For this review, take the finished solid that the model builds, in its own axes (mm). A direction names the side the tool comes from. Give positions to 0.01 mm unless a question says otherwise; leave off trailing zeros. Order: outer loops, then holes, each group sorted by start corner. A loop starts at its lowest first (then second) coordinate and runs counter-clockwise, first axis right, second up. Notation, with made-up numbers: (43, 53.25) -> (54, 53.25) arc R5 ccw to (54, 60.25) -> close; hole circle Ø10 at (-22.5, -24.5). An arc over 180 degrees is marked (long way). Return JSON: item names as keys, results as strings. Group by question number.
1) Add section D-D (x = 123). Give the boundary of the cut face in (y, z).
2) Add section B-B (x = -110). Give the boundary of the cut face in (y, z), then the cut area to 3 significant figures.
3) Add section A-A (z = 196). Give the boundary of the cut face in (x, y), then the cut area to 3 significant figures.
4) To check wall thickness, follow line 1 along Z through (x, y) = (18.5, 234); line 2 along Z through (x, y) = (100.5, 329); line 3 along Y through (x, z) = (327.5, 166). State the ranges of each line that lie inside material, in increasing order.
5) The part is to be moulded in two halves that separate along X. For faces 4 (the face through (211, 309, 0)), 5 (the face through (104.15, -180.39, 138.19)), 6 (the face through (487.348, 444.111, 118.11)), say which applies: released by +X, released by -X, zero draft, split by the parting line, or undercut.
6) Add section C-C (y = 546.5). Give the boundary of the cut face in (x, z), then the cut area to 3 significant figures.
7) Insertion check: P1, Ø12, axis at x = 323, z = 144.5, coming from the +Y side; P2, Ø16, axis at y = 202.5, z = 289, coming from the -X side; P3, Ø2, axis at x = 314.5, z = 206, coming from the -Y side. Each pin has a flat end and moves straight along its axis. Give the tip position at first contact, or say it passes through.
8) For faces 1 (the face through (-108, 345, 148)), 2 (the face through (-111, 424, 270)), 3 (the face through (0, 474, 148)), list the 3-axis set-ups (+Z, -Z, +X, -X, +Y, -Y) from which the entire face can be reached by the end or side of a thin tool; tool diameter is ignored.
from build123d import *

# Parameters (mm, degrees)
BOSS_EXTRUDE1_DEPTH = 300
CUT_EXTRUDE2_START  = -20
CUT_EXTRUDE2_DEPTH  = 260
SKETCH3_R           = 25
CUT_EXTRUDE3_DEPTH  = 932.86425071
SKETCH4_R           = 15
SKETCH4_W           = 55
SKETCH4_H           = 160
CUT_EXTRUDE4_DEPTH  = 932.86425071
SKETCH5_R           = 15
SKETCH5_W           = 160
SKETCH5_H           = 55
CUT_EXTRUDE5_DEPTH  = 1055.203993494
SKETCH7_R           = 15
SKETCH7_W           = 55
SKETCH7_H           = 160
CUT_EXTRUDE6_DEPTH  = 954.980428731
CUT_EXTRUDE7_REACH  = 933.864
SKETCH8_R           = 110
SKETCH9_W           = 270
SKETCH9_H           = 190
CUT_EXTRUDE8_DEPTH  = 100
CIRPATTERN1_COUNT   = 3


with BuildPart() as part:
    # Sketch1 → Boss-Extrude1 (new body)
    with BuildSketch(Plane.XY):
        Polygon((0, 0), (0, 345), (-220, 345), (-220, 600), (0, 600), (298.778764306, 427.5), (408.778764306, 618.025588833), (629.615242271, 490.525588833), (519.615242271, 300), (220.836477965, 127.5), (330.836477965, -63.025588833), (110, -190.525588833), align=None)
    extrude(amount=BOSS_EXTRUDE1_DEPTH)

    # Sketch2 → Cut-Extrude2 (cut)
    with BuildSketch(Plane(origin=(0, 0, 0), x_dir=(-1, 0, 0), z_dir=(0, 0, -1)).offset(CUT_EXTRUDE2_START)):
        Polygon((0, 600), (0, 0), (-519.615242271, 300), align=None)
    extrude(amount=-CUT_EXTRUDE2_DEPTH, mode=Mode.SUBTRACT)

    # Sketch3 → Cut-Extrude3 (cut, through all)
    with BuildSketch(Plane(origin=(0, 0, 0), x_dir=(-1, 0, 0), z_dir=(0, 0, -1))):
        with Locations((-173.205080757, 300)):
            Circle(SKETCH3_R)
    extrude(amount=-CUT_EXTRUDE3_DEPTH, mode=Mode.SUBTRACT)

    # Sketch4 → Cut-Extrude4 (cut, through all)
    with BuildSketch(Plane(origin=(0, 0, 0), x_dir=(0, 0, 1), z_dir=(-0.866025403784456, -0.4999999999999701, 0))):
        with Locations(Location((100, -110, 0), (0, 0, 270))):
            Circle(SKETCH4_R)
        with Locations((242.5, -110)):
            Rectangle(SKETCH4_W, SKETCH4_H)
    extrude(amount=-CUT_EXTRUDE4_DEPTH, mode=Mode.SUBTRACT)

    # Sketch5 → Cut-Extrude5 (cut, through all)
    with BuildSketch(Plane(origin=(0, 600, 0), x_dir=(1, 0, 0), z_dir=(0, 1, 0))):
        with Locations(Location((-110, -100, 0), (0, 0, 180))):
            Circle(SKETCH5_R)
        with Locations((-110, -242.5)):
            Rectangle(SKETCH5_W, SKETCH5_H)
    extrude(amount=-CUT_EXTRUDE5_DEPTH, mode=Mode.SUBTRACT)

    # Sketch7 → Cut-Extrude6 (cut, through all)
    with BuildSketch(Plane(origin=(259.807621135, -150, 0), x_dir=(0, 0, -1), z_dir=(0.8660254037844342, -0.5000000000000079, 0))):
        with Locations(Location((-100, 629.615242271, 0), (0, 0, 90))):
            Circle(SKETCH7_R)
        with Locations((-242.5, 629.615242271)):
            Rectangle(SKETCH7_W, SKETCH7_H)
    extrude(amount=-CUT_EXTRUDE6_DEPTH, mode=Mode.SUBTRACT)

    # Sketch8 → Cut-Extrude7 (cut, up to next)
    with BuildSketch(Plane.XY.offset(300), mode=Mode.PRIVATE) as cut_extrude7_sk1:
        with Locations((173.205080757, 300)):
            Circle(SKETCH8_R)
    cut_extrude7_tool1 = extrude(cut_extrude7_sk1.sketch, amount=-CUT_EXTRUDE7_REACH, mode=Mode.PRIVATE) & part.part
    add(cut_extrude7_tool1.solids().sort_by_distance((173.205081, 300, 300))[0], mode=Mode.SUBTRACT)

    # Sketch9 → Cut-Extrude8 (cut)
    with BuildSketch(Plane(origin=(0, 0, 0), x_dir=(0, 0, 1), z_dir=(-0.866025403784456, -0.4999999999999701, 0))):
        with Locations((150, -110)):
            Rectangle(SKETCH9_W, SKETCH9_H)
    cut_extrude8 = extrude(amount=-CUT_EXTRUDE8_DEPTH, mode=Mode.SUBTRACT)

    # CirPattern1: Cut-Extrude8 ×3 about axis
    cirpattern1_axis = Axis((173.205080757, 300, 0), (0, 0, 1))
    for i in range(1, CIRPATTERN1_COUNT):
        add(cut_extrude8.rotate(cirpattern1_axis, i * 360 / CIRPATTERN1_COUNT), mode=Mode.SUBTRACT)


solid = part.part
Evaluation:
{
 "1": {"outline": "(-183.02, 0) -> (528.99, 0) -> (528.99, 20) -> (71.01, 20) -> (71.01, 280) -> (202.13, 280) -> (202.13, 300) -> (-183.02, 300) -> close; (397.87, 280) -> (528.99, 280) -> (528.99, 300) -> (397.87, 300) -> close; hole (-165.7, 15) -> (-13.04, 15) -> (-13.04, 215) -> (36.37, 215) -> (36.37, 270) -> (-13.04, 270) -> (-13.04, 285) -> (-165.7, 285) -> close"},
 "2": {"outline": "(345, 0) -> (600, 0) -> (600, 15) -> (500, 15) -> (500, 85) -> (345, 85) -> close; (345, 115) -> (500, 115) -> (500, 215) -> (345, 215) -> close; (345, 270) -> (500, 270) -> (500, 285) -> (600, 285) -> (600, 300) -> (345, 300) -> close", "area": "36,300 mm^2"},
 "3": {"outline": "(-220, 345) -> (0, 345) -> (0, 600) -> (-15, 600) -> (-15, 500) -> (-205, 500) -> (-205, 600) -> (-220, 600) -> close; (0, 0) -> (7.5, -12.99) -> (94.1, 37.01) -> (189.1, -127.54) -> (102.5, -177.54) -> (110, -190.53) -> (330.84, -63.03) -> (220.84, 127.5) -> close; (298.78, 427.5) -> (519.62, 300) -> (527.12, 312.99) -> (440.51, 362.99) -> (535.51, 527.54) -> (622.12, 477.54) -> (629.62, 490.53) -> (408.78, 618.03) -> close", "area": "111,000 mm^2"},
 "4": {"line 1": "0 to 20, 280 to 300", "line 2": "0 to 20", "line 3": "-64.95 to -57.25, 410.92 to 477.25"},
 "5": {"face 4": "zero draft", "face 5": "released by -X", "face 6": "undercut"},
 "6": {"outline": "(-220, 0) -> (92.66, 0) -> (92.66, 20) -> (0, 20) -> (0, 280) -> (92.66, 280) -> (92.66, 300) -> (-220, 300) -> close; (367.48, 0) -> (532.66, 0) -> (532.66, 300) -> (367.48, 300) -> (367.48, 270) -> (472.66, 270) -> (472.66, 215) -> (367.48, 215) -> close; hole (-205, 15) -> (-15, 15) -> (-15, 285) -> (-205, 285) -> close", "area": "62,200 mm^2"},
 "7": {"P1": "y = 479.84", "P2": "x = 0", "P3": "y = -73.03"},
 "8": {"face 1": "+Z, -Z, -X, -Y", "face 2": "+Y, -Y", "face 3": "+Y"}
}
